Check sheet for the drawn part. Datum: minimum x, y, z corner. Units: mm. A direction names the side the tool comes from. Coordinates: 2 decimals unless noted, no trailing zeros. Order: outer loops, then holes, each group sorted by start corner. A loop starts at its lowest first (then second) coordinate and runs counter-clockwise, first axis right, second up. Notation, with made-up numbers: (49.5, 12) -> (54.5, 12) arc R26 ccw to (54.5, 50) -> close; hole circle Ø11 at (66, -37). An arc over 180 degrees is marked (long way). Answer as CSV lines item,"result".
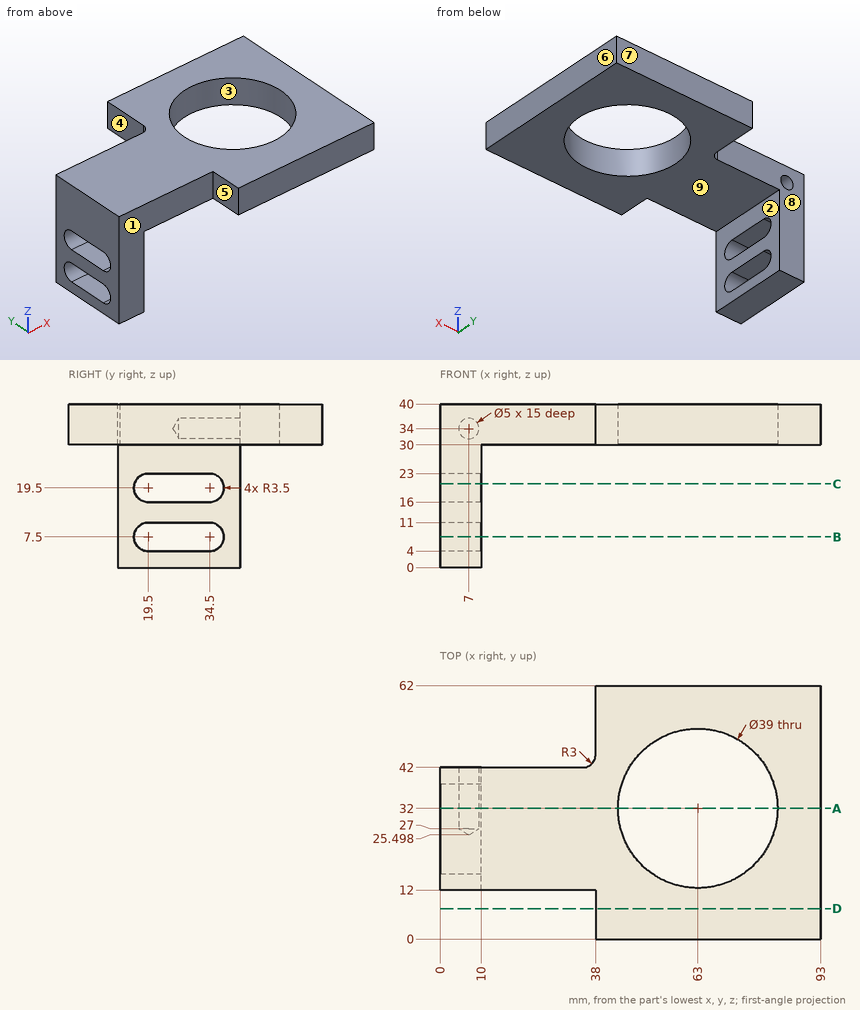
Item 1: Tool access check on the marked faces 5, 6, 7, 8 and 9. Record the directions out of +Z, -Z, +X, -X, +Y, -Y that give a thin tool (end or side, any length) a straight path to the whole face; none if there is none.
Answer list:
face 5,"+Z, -Z, -X, -Y"
face 6,"+Z, -Z, +X, +Y, -Y"
face 7,"+Z, -Z, +X, -X, +Y"
face 8,"+Z, -Z, -X, +Y"
face 9,"-Z, +X, +Y, -Y"
Item 2: Depth check by flat-ended pin: pin 1 Ø8 at (x, y) = (33, 10) entering from -Z; pin 2 Ø11 at (y, z) = (4.5, 35) entering from -X; pin 3 Ø3 at (x, z) = (7, 34) entering from -Y; pin 4 Ø23.5 at (x, y) = (63, 32) entering from +Z. Enter the tip coordinate at first touch or a pass-through.
Answer list:
pin 1,"z = 30"
pin 2,"x = 38"
pin 3,"y = 12"
pin 4,"through"
Item 3: Release check for a two-part mould opening along X. For the marked faces 1, 2, 3 and 4 record: +X half, -X half, draft (parallel to the pull), parting line (faces both ways), or undercut.
Answer list:
face 1,"draft"
face 2,"+X half"
face 3,"undercut"
face 4,"-X half"
Item 4: Section check B-B, the plane z = 7.5. Record the boundary of the cut face in (x, y), plus the area to 3 significant figures.
Answer list:
outline,"(0, 12) -> (10, 12) -> (10, 16) -> (0, 16) -> close; (0, 38) -> (10, 38) -> (10, 42) -> (0, 42) -> close"
area,"80.0 mm2"
Item 5: Section check A-A, the plane y = 32. Record the boundary of the cut face in (x, z), plus the area to 3 significant figures.
Answer list:
outline,"(0, 0) -> (10, 0) -> (10, 4) -> (0, 4) -> close; (0, 11) -> (10, 11) -> (10, 16) -> (0, 16) -> close; (0, 23) -> (10, 23) -> (10, 30) -> (43.5, 30) -> (43.5, 40) -> (0, 40) -> close; (82.5, 30) -> (93, 30) -> (93, 40) -> (82.5, 40) -> close; hole circle Ø5 at (7, 34)"
area,"680 mm2"
Item 6: Section check C-C, the plane z = 20.5. Record the boundary of the cut face in (x, y).
Answer list:
outline,"(0, 12) -> (10, 12) -> (10, 16.15) -> (0, 16.15) -> close; (0, 37.85) -> (10, 37.85) -> (10, 42) -> (0, 42) -> close"
Item 7: Thickness scan on line 1 (X direction, y = 37.75, z = 34); line 2 (X direction, y = 39.25, z = 34); line 3 (Z direction, x = 22.5, y = 37.5). Record the ranges inside material, lowest first.
Answer list:
line 1,"0 to 4.5, 9.5 to 44.37, 81.63 to 93"
line 2,"0 to 4.5, 9.5 to 44.9, 81.1 to 93"
line 3,"30 to 40"
Item 8: Section check D-D, the plane y = 7.5. Record the boundary of the cut face in (x, z), plus the area to 3 significant figures.
Answer list:
outline,"(38, 30) -> (93, 30) -> (93, 40) -> (38, 40) -> close"
area,"550 mm2"
